from build123d import *

# Parameters (mm, degrees)
SKETCH2_R           = 130
SKETCH2_R_2         = 27.5
BOSS_EXTRUDE1_DEPTH = 15
SKETCH3_R           = 10
CUT_EXTRUDE1_DEPTH  = 185.458667457
CIRPATTERN1_COUNT   = 8


with BuildPart() as part:
    # Sketch2 → Boss-Extrude1 (new body)
    with BuildSketch(Plane.XY):
        Circle(SKETCH2_R)
        Circle(SKETCH2_R_2, mode=Mode.SUBTRACT)
    extrude(amount=BOSS_EXTRUDE1_DEPTH)

    # Sketch3 → Cut-Extrude1 (cut, symmetric)
    with BuildSketch(Plane.XY):
        with Locations((-115, 0)):
            Circle(SKETCH3_R)
    cut_extrude1 = extrude(amount=CUT_EXTRUDE1_DEPTH, both=True, mode=Mode.SUBTRACT)

    # CirPattern1: Cut-Extrude1 ×8 about axis
    cirpattern1_axis = Axis((0, 0, 0), (0, 0, 1))
    for i in range(1, CIRPATTERN1_COUNT):
        add(cut_extrude1.rotate(cirpattern1_axis, i * 360 / CIRPATTERN1_COUNT), mode=Mode.SUBTRACT)


solid = part.part
Build history of the part. All positions in model axes, mm. Give positions to 0.01 mm unless a question says otherwise; leave off trailing zeros. Order: outer loops, then holes, each group sorted by start corner. A loop starts at its lowest first (then second) coordinate and runs counter-clockwise, first axis right, second up. Notation, with made-up numbers: M -24,-17 L 29,-17 A13 cw 29,2 Z; hole C 60,-15 d10. An arc over 180 degrees is marked long. Put each result on its own line as item: value.
Item 1: Pull direction Y, two halves, no side cores. Call faces 1 (the face through (123.997, 39.048, 7.395)), 2 (the face through (-2, 31, 0)), 3 (the face through (0, 125, 8)): +Y half, -Y half, draft (parallel to the pull), parting line (faces both ways), or undercut.
Results are:
face 1: parting line
face 2: draft
face 3: undercut
Item 2: Cut at B-B on x = -115. Write the cut outline in (y, z).
Results are:
outline: M -60.62,0 L -10,0 L -10,15 L -60.62,15 Z; M 10,0 L 60.62,0 L 60.62,15 L 10,15 Z
Item 3: Cut at C-C on y = -113. Write the cut outline in (x, z).
Results are:
outline: M -64.27,0 L -9.8,0 L -9.8,15 L -64.27,15 Z; M 9.8,0 L 64.27,0 L 64.27,15 L 9.8,15 Z
Item 4: Wall check: probe 1 along X at (y, z) = (1, 11.75); probe 2 along X at (y, z) = (4, 2.5); probe 3 along Y at (x, z) = (-77, 11.5). Give the ranges that are in metal, low to high.
Results are:
probe 1: -130 to -124.95, -105.05 to -27.48, 27.48 to 105.05, 124.95 to 130
probe 2: -129.94 to -124.17, -105.83 to -27.21, 27.21 to 105.83, 124.17 to 129.94
probe 3: -104.74 to -90.34, -72.3 to 72.3, 90.34 to 104.74
Item 5: Drop flat-ended pins along their axis: pin 1 Ø3 at (x, z) = (-103, 12.5) entering from -Y; pin 2 Ø6 at (y, z) = (34, 6) entering from -X; pin 3 Ø3 at (x, z) = (-100, 8) entering from -Y. Give the stop position or say it passes through.
Results are:
pin 1: y = -81.23
pin 2: x = -126.25
pin 3: y = -84.84
Item 6: Cut at A-A on y = 0. Write the cut outline in (x, z).
Results are:
outline: M -130,0 L -125,0 L -125,15 L -130,15 Z; M -105,0 L -27.5,0 L -27.5,15 L -105,15 Z; M 27.5,0 L 105,0 L 105,15 L 27.5,15 Z; M 125,0 L 130,0 L 130,15 L 125,15 Z
Item 7: Cut at D-D on z = 5. Count the separate pieces of the cut face and the enclosed holes in it, then the cut area to 3 significant figures.
Results are:
separate pieces: 1
enclosed holes: 9
area: 48,200 mm2
